```python
from build123d import *

# Parameters (mm, degrees)
EXTRUDE_1_DEPTH = 8
CHAMFER_1_SIZE  = 20


with BuildPart() as part:
    # 草图2 → 凸台-拉伸1 (new, symmetric)
    with BuildSketch(Plane.XY):
        Polygon((0, 0), (42, 695), (137, 695), (137, 0), align=None)
    extrude(amount=EXTRUDE_1_DEPTH, both=True)

    # 倒角1
    chamfer_1_edges = [part.edges().sort_by_distance(p)[0] for p in [
        (137, 695, 0),
        (137, 0, 0),
    ]]
    chamfer(chamfer_1_edges, length=CHAMFER_1_SIZE)


solid = part.part
```
Source: CAD feature listing. Evaluate the final solid. Frame: model axes, mm. Give positions to 0.01 mm unless a question says otherwise; leave off trailing zeros. Order: outer loops, then holes, each group sorted by start corner. A loop starts at its lowest first (then second) coordinate and runs counter-clockwise, first axis right, second up.
(1) Contact query for a flat-ended pin moving along its axis: P1, Ø2, axis at x = 119.5, z = 5, coming from the +Y side. Output: stop coordinate, or through.
(2) Material intervals for line 1 along X through (y, z) = (515, -2); line 2 along X through (y, z) = (292, 0); line 3 along Y through (x, z) = (120, 4), sorted ascending.
(3) Section query B-B (x = 125). Return the cut outline in (y, z).
(4) Section query A-A (z = -1.75). Return the cut outline in (x, y).
(5) Section query C-C (y = 395). Return the cut outline in (x, z), plus the area to 3 significant figures.
Outcome:
1. P1: stops at y = 693.5
2. line 1: x = 31.12 to 137
2. line 2: x = 17.65 to 137
2. line 3: y = 3 to 692
3. outline: (8, -8) - (687, -8) - (687, 8) - (8, 8) - close
4. outline: (0, 0) - (117, 0) - (137, 20) - (137, 675) - (117, 695) - (42, 695) - close
5. outline: (23.87, -8) - (137, -8) - (137, 8) - (23.87, 8) - close
5. area: 1,810 mm2
